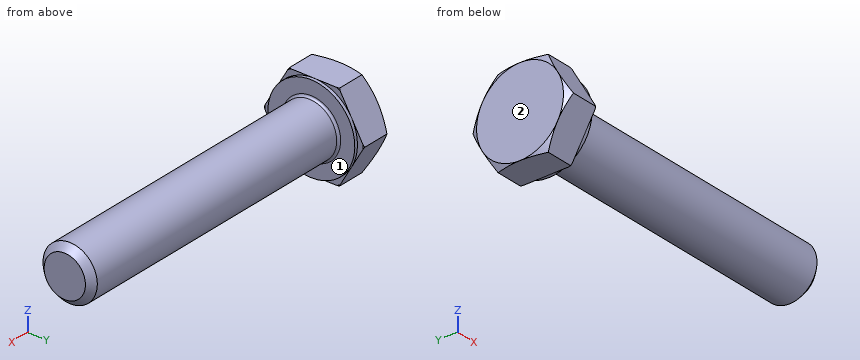
from build123d import *

# Parameters (mm, degrees)
EXTRUDE_371_DEPTH = 6.4
SKETCH_4_W        = 0.6
SKETCH_4_H        = 11.237604307
CHAMFER_2038_SIZE = 1.2
FILLET_2080_R     = 0.4


with BuildPart() as part:
    # 草图1 → Extrude 371 (new body)
    with BuildSketch(Plane(origin=(0, 0, 0), x_dir=(0, 0, -1), z_dir=(1, 0, 0))):
        Polygon((8, 4.618802154), (8, -4.618802154), (0, -9.237604307), (-8, -4.618802154), (-8, 4.618802154), (0, 9.237604307), align=None)
    extrude(amount=EXTRUDE_371_DEPTH)

    # 草图2 → 凸台-旋转1 (revolve)
    with BuildSketch(Plane.XY, mode=Mode.PRIVATE) as revolve_1_sk:
        Polygon((0, 0), (61.4, 0), (61.4, 3.701), (61.4, 5), (27.8072, 5), (0, 5), align=None)
    revolve(revolve_1_sk.sketch.rotate(Axis((0, 0, 0), (1, 0, 0)), 90), axis=Axis((0, 0, 0), (1, 0, 0)))

    # 草图3 → 切除-旋转1 (revolve, cut)
    with BuildSketch(Plane.XY):
        Polygon((0, 8), (3.601282526, 14.237604307), (3.601282526, 19.237604307), (-10, 19.237604307), (-10, 8), align=None)
    revolve(axis=Axis((0, 0, 0), (1, 0, 0)), mode=Mode.SUBTRACT)

    # 草图5 → 切除-旋转2 (revolve, cut)
    with BuildSketch(Plane.XY):
        Polygon((6.4, 8), (2.798717474, 14.237604307), (2.798717474, 19.237604307), (12.798717474, 19.237604307), (12.798717474, 8), align=None)
    revolve(axis=Axis((0, 0, 0), (1, 0, 0)), mode=Mode.SUBTRACT)

    # 草图4 → 切除-旋转3 (revolve, cut)
    with BuildSketch(Plane.XY, mode=Mode.PRIVATE) as cut_revolve_3_sk:
        with Locations((6.1, 13.618802154)):
            Rectangle(SKETCH_4_W, SKETCH_4_H)
    revolve(cut_revolve_3_sk.sketch.rotate(Axis((0, 0, 0), (1, 0, 0)), 270), axis=Axis((0, 0, 0), (1, 0, 0)), mode=Mode.SUBTRACT)

    # Chamfer 2038
    chamfer_2038_edges = [part.edges().sort_by_distance(p)[0] for p in [
        (61.4, 0, -5),
    ]]
    chamfer(chamfer_2038_edges, length=CHAMFER_2038_SIZE)

    # Fillet 2080
    fillet_2080_edges = [part.edges().sort_by_distance(p)[0] for p in [
        (6.4, 0, -5),
    ]]
    fillet(fillet_2080_edges, radius=FILLET_2080_R)


solid = part.part
Work out the finished part from the listing and answer in its coordinate system (mm). Face numbers are marked on the shaded views. A direction names the side the tool comes from. Give positions to 0.01 mm unless a question says otherwise; leave off trailing zeros. Loops run counter-clockwise (first coordinate to the right, second up) from the corner with the lowest first, then second, coordinate; pieces in that order, holes last. Notation, with made-up numbers: (-11.75, 44) -> (11.25, 44) arc R29 cw to (11.25, 66) -> close; hole circle Ø9 at (66, -23). An arc over 180 degrees is marked (long way). Use a Markdown table: item, result. Add a question column.
1) The part is cut by section A-A, the plane x = 32. Determine the outline of the cut face in (y, z).
2) Each of these flat-tipped pins is pushed along its axis until it touches: P1, Ø3, axis at x = 50.5, z = -0.5, coming from the +Y side; P2, Ø4, axis at x = 47, z = -5.5, coming from the -Y side; P3, Ø4.5, axis at y = -4, z = 5.5, coming from the +X side. Where does it stop, or does it pass through?
3) Consider line 1 along X through (y, z) = (-7.25, -2); line 2 along Z through (x, y) = (6.5, -2.5); line 3 along Y through (x, z) = (39, 0.25). Determine where each line is inside the solid, lowest interval first.
4) Which of the six approach directions +Z, -Z, +X, -X, +Y, -Y give full straight-line access (tool end or side, diameter ignored) to the marked faces 1 and 2?
Reported:
| question | item | result |
|---|---|---|
| 1 | outline | circle Ø10 at (0, 0) |
| 2 | P1 | stops at y = 5 |
| 2 | P2 | stops at y = -3.57 |
| 2 | P3 | stops at x = 60.65 |
| 3 | line 1 | x = 0 to 6.4 |
| 3 | line 2 | z = -4.49 to 4.49 |
| 3 | line 3 | y = -4.99 to 4.99 |
| 4 | face 1 | +X |
| 4 | face 2 | +Z, -Z, -X, +Y, -Y |
